from build123d import *
from OCP.BRepFilletAPI import BRepFilletAPI_MakeChamfer

# Parameters (mm, degrees)
SKETCH1_W           = 320
SKETCH1_H           = 80
BOSS_EXTRUDE1_DEPTH = 55
CUT_EXTRUDE1_DEPTH  = 188.149672722
CUT_EXTRUDE2_DEPTH  = 188.149672722
SKETCH7_R           = 6.5
CUT_EXTRUDE3_DEPTH  = 169.597153001
CHAMFER1_SIZE       = 3
CHAMFER1_SIZE2      = 2.154045129


with BuildPart() as part:
    # Sketch1 → Boss-Extrude1 (new body)
    with BuildSketch(Plane(origin=(0, 0, 0), x_dir=(1, 0, 0), z_dir=(0, 1, 0))):
        Rectangle(SKETCH1_W, SKETCH1_H)
    extrude(amount=BOSS_EXTRUDE1_DEPTH)

    # Sketch2 → Cut-Extrude1 (cut, through all)
    with BuildSketch(Plane.XY.offset(40)):
        Polygon((105.068765597, 55), (128.585786438, 21.414213562), (130, 20), (128.585786438, 18.585786438), (127.171572875, 20), (70, 20), (68, 18), (-43, 18), (-45, 20), (-128.585786438, 20), (-130, 18.585786438), (-131.414213562, 20), (-130, 21.414213562), (-130, 55), align=None)
    extrude(amount=-CUT_EXTRUDE1_DEPTH, mode=Mode.SUBTRACT)

    # Sketch3 → Cut-Extrude2 (cut, through all)
    with BuildSketch(Plane.XY.offset(40)):
        Polygon((-26.085786438, 3), (26.085786438, 3), (27.5, 4.414213562), (28.914213562, 3), (27.5, 1.585786438), (27.5, 0), (-27.5, 0), (-27.5, 1.585786438), (-28.914213562, 3), (-27.5, 4.414213562), align=None)
    extrude(amount=-CUT_EXTRUDE2_DEPTH, mode=Mode.SUBTRACT)

    # Sketch6 → M8 Tapped Hole1 (revolve, cut)
    with BuildSketch(Plane(origin=(17.5, 3, -27.5), x_dir=(0, 0, -1), z_dir=(1, 0, 0))):
        Polygon((0, 0), (0, 21.792926105), (3.4, 19.75), (3.4, 0.625), (4.025, 0), align=None)
    m8_tapped_hole1 = revolve(axis=Axis((17.5, -3.35, -27.5), (0, 1, 0)), mode=Mode.SUBTRACT)

    # Mirror1: M8 Tapped Hole1 across plane
    add(m8_tapped_hole1.mirror(Plane(origin=(0, 0, 0), x_dir=(0, 0, 1), z_dir=(1, 0, 0))), mode=Mode.SUBTRACT)

    # Mirror2: M8 Tapped Hole1 across plane
    add(m8_tapped_hole1.mirror(Plane.XY), mode=Mode.SUBTRACT)

    # Mirror2 copy 1 sketch → Mirror2 copy 1 (revolve, cut)
    with BuildSketch(Plane(origin=(-17.5, 3, 27.5), x_dir=(0, 0, 1), z_dir=(-1, 0, 0))):
        Polygon((0, 0), (0, 21.792926105), (3.4, 19.75), (3.4, 0.625), (4.025, 0), align=None)
    revolve(axis=Axis((-17.5, -3.35, 27.5), (0, 1, 0)), mode=Mode.SUBTRACT)

    # Sketch7 → Cut-Extrude3 (cut, through all)
    with BuildSketch(Plane(origin=(0, 20, 0), x_dir=(1, 0, 0), z_dir=(0, 1, 0))):
        with Locations(Location((-119, 27.5, 0), (0, 0, 270))):
            Circle(SKETCH7_R)
        with Locations(Location((-119, -27.5, 0), (0, 0, 90))):
            Circle(SKETCH7_R)
    extrude(amount=-CUT_EXTRUDE3_DEPTH, mode=Mode.SUBTRACT)

    # Chamfer1: one chamfer whose edges measure the first distance from different faces: ONE call of the kernel's chamfer builder (chamfer() names one face for all edges)
    chamfer1_edges_1 = [part.edges().sort_by_distance(p)[0] for p in [
        (-160, 55, 0),
        (160, 55, 0),
        (-160, 0, 0),
        (160, 0, 0),
    ]]
    chamfer1_edges_2 = [part.edges().sort_by_distance(p)[0] for p in [
        (105.068765597, 55, 0),
    ]]
    chamfer1_side_2 = [part.faces().sort_by_distance(p)[0] for p in [
        (116.827276017, 38.207106781, 0),
    ]]
    chamfer1 = BRepFilletAPI_MakeChamfer(part.part.solid().wrapped)
    for e in chamfer1_edges_1:
        chamfer1.Add(CHAMFER1_SIZE, e.wrapped)
    for e in chamfer1_edges_2:
        chamfer1.Add(CHAMFER1_SIZE, CHAMFER1_SIZE2, e.wrapped, chamfer1_side_2[0].wrapped)  # the first distance lies on this face
    add(Compound.cast(chamfer1.Shape()), mode=Mode.REPLACE)


solid = part.part
Model file for the job. Use its own axes, mm. A direction names the side the tool comes from. Give positions to 0.01 mm unless a question says otherwise; leave off trailing zeros. Order: outer loops, then holes, each group sorted by start corner. A loop starts at its lowest first (then second) coordinate and runs counter-clockwise, first axis right, second up. Notation, with made-up numbers: M 16,-6.5 L 44,-6.5 A38 cw 44,32.5 Z; hole C 39,9.5 d4. An arc over 180 degrees is marked long. Put each result on its own line as item: value. Start each with the question number.
(1) Tool access for faces 5 (the face through (-160, 27, 1)), 6 (the face through (-130, 38, 1)): list every direction of +Z, -Z, +X, -X, +Y, -Y with a clear straight run to the whole face (end or side of a thin tool).
(2) Pin check, flat tips, straight feed: pin 1 Ø1.3 at (y, z) = (1, -11) entering from -X; pin 2 Ø1.5 at (x, z) = (54.5, -10.5) entering from +Y; pin 3 Ø11.5 at (x, z) = (-119, -27.5) entering from -Y; pin 4 Ø0.8 at (y, z) = (0.5, -18.5) entering from +X. Stop position of each tip, or through.
(3) Pull direction X, two halves, no side cores. Call faces 1 (the face through (99, 20, 1)), 2 (the face through (0, 3, 1)), 3 (the face through (132, 55, -1)), 4 (the face through (160, 27, 1)): released by +X, released by -X, zero draft, split by the parting line, or undercut.
(4) Drill centre lines: L1, parallel to X at y = 11, z = 27; L2, parallel to Z at x = -17, y = 12; L3, parallel to X at y = 4, z = 16. Where is each one in solid material? Low to high. Write a range as [from, to].
(5) Band-saw the part on A-A on x = -17.5. Give the cut face in (y, z) (3 decimals).
(6) Band-saw the part on B-B on y = 38.5. Give the cut face in (x, z).
(7) Band-saw the part on C-C on z = 27.5. Count the separate pieces of the cut face and the enclosed holes in it, then the cut area to 3 significant figures.
Results below:
1. face 5: +Z, -Z, -X, +Y, -Y
1. face 6: +Z, -Z, +Y
2. pin 1: stops at x = -158.65
2. pin 2: stops at y = 18
2. pin 3: passes through
2. pin 4: stops at x = 157.9
3. face 1: undercut
3. face 2: undercut
3. face 3: zero draft
3. face 4: released by +X
4. L1: x = [-160, -125.48], [-112.52, -20.86], [-14.14, 14.14], [20.86, 160]
4. L2: z = [-40, -30.86], [-24.14, 24.14], [30.86, 40]
4. L3: x = [-160, -27.91], [-27.09, 27.09], [27.91, 160]
5. outline: M 3,-40 L 18,-40 L 18,-30.9 L 3.625,-30.9 L 3,-31.525 Z; M 3,-23.475 L 3.625,-24.1 L 18,-24.1 L 18,24.1 L 3.625,24.1 L 3,23.475 Z; M 3,31.525 L 3.625,30.9 L 18,30.9 L 18,40 L 3,40 Z
6. outline: M -160,-40 L -130,-40 L -130,40 L -160,40 Z; M 116.62,-40 L 160,-40 L 160,40 L 116.62,40 Z
7. separate pieces: 4
7. enclosed holes: 0
7. area: 8,060 mm2
